Part print with two shaded views. Sizes in mm from the minimum x, y, z corner. A direction names the side the tool comes from. Round coordinates to 2 decimals unless told otherwise and drop trailing zeros. Write each loop counter-clockwise with the first axis right and the second up, starting at its lowest first coordinate (ties: lowest second). Pieces come first, ordered by that corner, then holes.
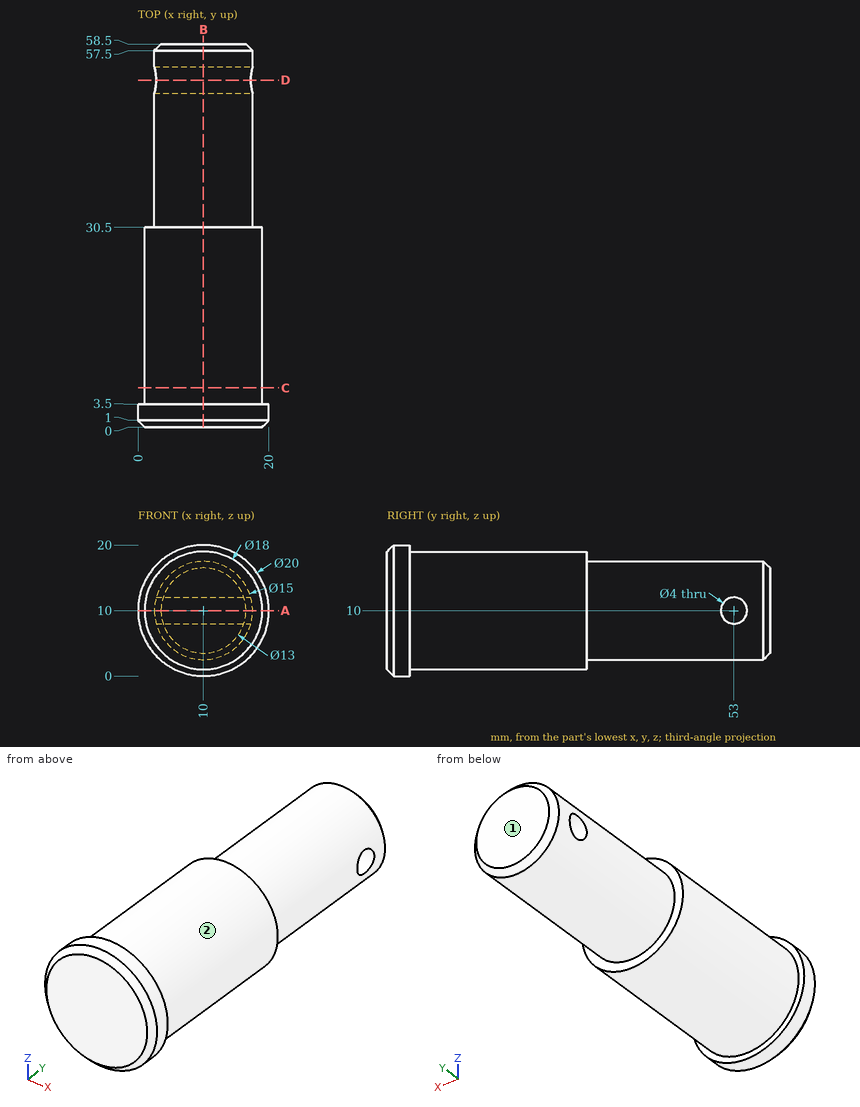
Q1. Drop flat-ended pins along their axis: pin 1 (4 mm diameter, centred on y = 35.5, z = 12.5, fed in from +X); pin 2 (8 mm diameter, centred on y = 12, z = 13, fed in from -X); pin 3 (2 mm diameter, centred on y = 51.5, z = 16.5, fed in from -X). Give the stop position or say it passes through.
Values follow:
pin 1: stops at x = 17.48
pin 2: stops at x = 1
pin 3: stops at x = 4.9
Q2. Cut at C-C on y = 6. Write the cut outline in (x, z), plus the area to 3 significant figures.
Values follow:
outline: circle Ø18 at (10, 10)
area: 254 mm2
Q3. Which spindle directions (+Z, -Z, +X, -X, +Y, -Y) get a long thin tool onto all of the face, cutting with end or side? Do the marked faces 1 and 2. Say none if no direction does.
Values follow:
face 1: +Z, -Z, +X, -X, +Y
face 2: +Y
Q4. Wall check: L1, parallel to Z at x = 10.5, y = 53; L2, parallel to Y at x = 6.5, z = 10.75; L3, parallel to Y at x = 6.75, z = 2. Give the ranges that are in metal, low to high.
Values follow:
L1: z = 2.52 to 8, 12 to 17.48
L2: y = 0 to 51.15, 54.85 to 58.5
L3: y = 0 to 30.5
Q5. Cut at B-B on x = 10. Write the cut outline in (y, z).
Values follow:
outline: (0, 1) - (1, 0) - (3.5, 0) - (3.5, 1) - (30.5, 1) - (30.5, 2.5) - (57.5, 2.5) - (58.5, 3.5) - (58.5, 16.5) - (57.5, 17.5) - (30.5, 17.5) - (30.5, 19) - (3.5, 19) - (3.5, 20) - (1, 20) - (0, 19) - close; hole circle Ø4 at (53, 10)
Q6. Cut at A-A on z = 10. Write the cut outline in (x, y), plus the area to 3 significant figures.
Values follow:
outline: (0, 1) - (1, 0) - (19, 0) - (20, 1) - (20, 3.5) - (19, 3.5) - (19, 30.5) - (17.5, 30.5) - (17.5, 51) - (2.5, 51) - (2.5, 30.5) - (1, 30.5) - (1, 3.5) - (0, 3.5) - close; (2.5, 55) - (17.5, 55) - (17.5, 57.5) - (16.5, 58.5) - (3.5, 58.5) - (2.5, 57.5) - close
area: 914 mm2
Q7. Cut at D-D on y = 53. Write the cut outline in (x, z), plus the area to 3 significant figures.
Values follow:
outline: (2.77, 8) arc R7.5 ccw to (17.23, 8) - close; (2.77, 12) - (17.23, 12) arc R7.5 ccw to start
area: 117 mm2
